from build123d import *

# Parameters (mm, degrees)
BASE_BLOCK_SKETCH_W           = 90
BASE_BLOCK_SKETCH_H           = 48
BASE_BLOCK_DEPTH              = 30
CHANNEL_SLOT_SKETCH_W         = 78
CHANNEL_SLOT_SKETCH_H         = 36
CHANNEL_SLOT_DEPTH            = 24
CHANNEL_RELIEF_CUT_1_SKETCH_W = 6
CHANNEL_RELIEF_CUT_1_SKETCH_H = 36
CHANNEL_RELIEF_CUT_1_DEPTH    = 24
CHANNEL_RELIEF_CUT_2_SKETCH_W = 6
CHANNEL_RELIEF_CUT_2_SKETCH_H = 36
CHANNEL_RELIEF_CUT_2_DEPTH    = 24
HALF_CYLINDER_BOSS_DEPTH      = 36
BOSS_BORE_18_DEPTH            = 42
UPPER_PLATE_HOLE_SKETCH_R     = 9
UPPER_PLATE_HOLE_18_DEPTH     = 6
LOWER_START                   = -6
LOWER_PLATE_HOLE_SKETCH_R     = 9
LOWER_PLATE_HOLE_18_DEPTH     = 6
C_CLIP_BOSS_DEPTH             = 20


with BuildPart() as part:
    # Base Block Sketch → Base Block (new body)
    with BuildSketch(Plane.XY):
        with Locations((45, 24)):
            Rectangle(BASE_BLOCK_SKETCH_W, BASE_BLOCK_SKETCH_H)
    extrude(amount=BASE_BLOCK_DEPTH)

    # Channel Slot Sketch → Channel Slot (cut)
    with BuildSketch(Plane.XY.offset(30)):
        with Locations((45, 24)):
            Rectangle(CHANNEL_SLOT_SKETCH_W, CHANNEL_SLOT_SKETCH_H)
    extrude(amount=-CHANNEL_SLOT_DEPTH, mode=Mode.SUBTRACT)

    # Channel Relief Cut 1 Sketch → Channel Relief Cut 1 (cut)
    with BuildSketch(Plane.XY.offset(30)):
        with Locations((3, 24)):
            Rectangle(CHANNEL_RELIEF_CUT_1_SKETCH_W, CHANNEL_RELIEF_CUT_1_SKETCH_H)
    extrude(amount=-CHANNEL_RELIEF_CUT_1_DEPTH, mode=Mode.SUBTRACT)

    # Channel Relief Cut 2 Sketch → Channel Relief Cut 2 (cut)
    with BuildSketch(Plane.XY.offset(30)):
        with Locations((87, 24)):
            Rectangle(CHANNEL_RELIEF_CUT_2_SKETCH_W, CHANNEL_RELIEF_CUT_2_SKETCH_H)
    extrude(amount=-CHANNEL_RELIEF_CUT_2_DEPTH, mode=Mode.SUBTRACT)

    # Half Cylinder Boss Sketch → Half Cylinder Boss (add)
    with BuildSketch(Plane.XY.offset(6)):
        with BuildLine():
            Line((0, 39), (0, 9))
            ThreePointArc((0, 9), (15, 24), (0, 39))
        make_face()
    extrude(amount=HALF_CYLINDER_BOSS_DEPTH)

    # Boss Bore Sketch → Boss Bore Ø18 (cut)
    with BuildSketch(Plane.XY.offset(42)):
        with BuildLine():
            Line((0, 33), (0, 15))
            ThreePointArc((0, 15), (9, 24), (0, 33))
        make_face()
    extrude(amount=-BOSS_BORE_18_DEPTH, mode=Mode.SUBTRACT)

    # Upper Plate Hole Sketch → Upper Plate Hole Ø18 (cut)
    with BuildSketch(Plane.XZ):
        with Locations(Location((45, 17, 0), (0, 0, 270))):
            Circle(UPPER_PLATE_HOLE_SKETCH_R)
    extrude(amount=-UPPER_PLATE_HOLE_18_DEPTH, mode=Mode.SUBTRACT)

    # Lower Plate Hole Sketch → Lower Plate Hole Ø18 (cut)
    with BuildSketch(Plane(origin=(0, 48, 0), x_dir=(1, 0, 0), z_dir=(0, 1, 0)).offset(LOWER_START)):
        with Locations(Location((45, -17, 0), (0, 0, 90))):
            Circle(LOWER_PLATE_HOLE_SKETCH_R)
    extrude(amount=LOWER_PLATE_HOLE_18_DEPTH, mode=Mode.SUBTRACT)

    # C Clip Boss Sketch → C Clip Boss (add)
    with BuildSketch(Plane.XY.offset(6)):
        Polygon((84, 35), (84, 29), (63, 29), (63, 19), (84, 19), (84, 13), (57, 13), (57, 35), align=None)
    extrude(amount=C_CLIP_BOSS_DEPTH)


solid = part.part
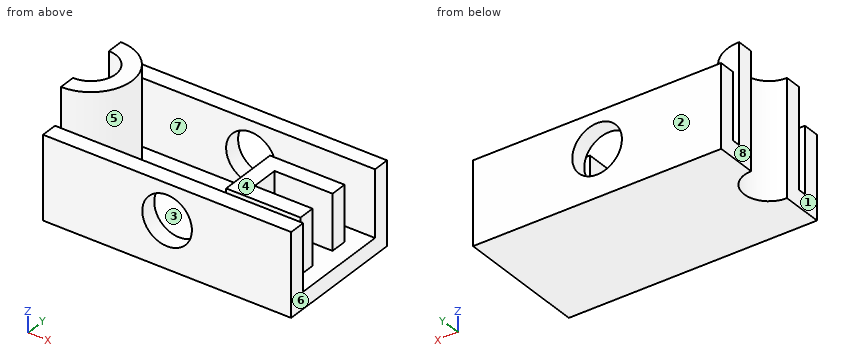
Read the model definition and answer for the solid it produces. Units are mm, in the model's axes. Face numbers are marked on the shaded views. A direction names the side the tool comes from. Round coordinates to 2 decimals unless told otherwise and drop trailing zeros. Write each loop counter-clockwise with the first axis right and the second up, starting at its lowest first coordinate (ties: lowest second). Pieces come first, ordered by that corner, then holes. Notation, with made-up numbers: (84, -24.5) - (94, -24.5) arc R21 cw to (94, 7.5) - close; hole circle Ø2 at (16, 48.5). An arc over 180 degrees is marked (long way). One line per question, with ' | ' between items. Start each with the question number.
1. Section C-C (x = 66.5) is taken. Determine the outline of the cut face in (y, z), and give its area (3 significant figures).
2. Section A-A (z = 17) is taken. Determine the outline of the cut face in (x, y).
3. Find the intervals of material crossed by probe 1 along X at (y, z) = (4, 17); probe 2 along Y at (x, z) = (70.5, 10.5); probe 3 along Y at (x, z) = (31, 7), in increasing order. Write a range as [from, to].
4. Section B-B (x = 45) is taken. Determine the outline of the cut face in (y, z), and give its area (3 significant figures).
5. For a pull along Y with two mould halves and no side action, classify the marked faces 1, 2 and 3 as +Y half, -Y half, draft (parallel to the pull), parting line (faces both ways), or undercut.
6. Each of these flat-tipped pins is pushed along its axis until it touches: pin 1 (4 mm diameter, centred on x = 71.5, y = 18, fed in from +Z); pin 2 (6.5 mm diameter, centred on x = 77, y = 24, fed in from +Z); pin 3 (6.5 mm diameter, centred on y = 33, z = 18, fed in from +X). Where does it stop, or does it pass through?
7. Section D-D (y = 24) is taken. Determine the outline of the cut face in (x, z), and give its area (3 significant figures).
8. For the marked faces 4, 5, 6, 7 and 8, determine the directions among +Z, -Z, +X, -X, +Y, -Y from which every point of the face is accessible in a straight line to the end or side of a thin tool.
Filled in:
1) outline: (0, 0) - (48, 0) - (48, 30) - (42, 30) - (42, 6) - (35, 6) - (35, 26) - (29, 26) - (29, 6) - (19, 6) - (19, 26) - (13, 26) - (13, 6) - (6, 6) - (6, 30) - (0, 30) - close | area: 816 mm²
2) outline: (0, 0) - (36, 0) - (36, 6) - (0, 6) - close; (0, 9) arc R15 ccw to (0, 39) - (0, 33) arc R9 cw to (0, 15) - close; (0, 42) - (36, 42) - (36, 48) - (0, 48) - close; (54, 0) - (90, 0) - (90, 6) - (54, 6) - close; (54, 42) - (90, 42) - (90, 48) - (54, 48) - close; (57, 13) - (84, 13) - (84, 19) - (63, 19) - (63, 29) - (84, 29) - (84, 35) - (57, 35) - close
3) probe 1: [0, 36], [54, 90] | probe 2: [0, 6], [13, 19], [29, 35], [42, 48] | probe 3: [0, 6], [42, 48]
4) outline: (0, 0) - (48, 0) - (48, 8) - (42, 8) - (42, 6) - (6, 6) - (6, 8) - (0, 8) - close; (0, 26) - (6, 26) - (6, 30) - (0, 30) - close; (42, 26) - (48, 26) - (48, 30) - (42, 30) - close | area: 360 mm²
5) face 1: draft | face 2: +Y half | face 3: undercut
6) pin 1: z = 26 | pin 2: z = 6 | pin 3: x = 84
7) outline: (9, 0) - (90, 0) - (90, 6) - (63, 6) - (63, 26) - (57, 26) - (57, 6) - (15, 6) - (15, 42) - (9, 42) - close | area: 822 mm²
8) face 4: +Z, +X | face 5: +Z | face 6: +Z, -Z, +X, +Y, -Y | face 7: +Z, +X, -X | face 8: +Z, -Z, -X, +Y, -Y
